Source: CAD feature listing. Evaluate the final solid. Frame: model axes, mm. Give positions to 0.01 mm unless a question says otherwise; leave off trailing zeros. Order: outer loops, then holes, each group sorted by start corner. A loop starts at its lowest first (then second) coordinate and runs counter-clockwise, first axis right, second up.
```python
from build123d import *

# Parameters (mm, degrees)
SKETCH1_W           = 100
SKETCH1_H           = 80
SKETCH1_R           = 2
BOSS_EXTRUDE1_DEPTH = 1


with BuildPart() as part:
    # Sketch1 → Boss-Extrude1 (new body)
    with BuildSketch(Plane.XY):
        Rectangle(SKETCH1_W, SKETCH1_H)
        with Locations((45, 36)):
            Circle(SKETCH1_R, mode=Mode.SUBTRACT)
        with Locations((-45, 36)):
            Circle(SKETCH1_R, mode=Mode.SUBTRACT)
        with Locations(Location((-45, -36, 0), (0, 0, 180))):
            Circle(SKETCH1_R, mode=Mode.SUBTRACT)
        with Locations(Location((45, -36, 0), (0, 0, 180))):
            Circle(SKETCH1_R, mode=Mode.SUBTRACT)
    extrude(amount=BOSS_EXTRUDE1_DEPTH)


solid = part.part
```
1) Draft query along Y for faces 1 (the flat face through (-1, 1, 1)), 2 (the cylindrical face through (-44.566, -34.048, 0.493)). Return one class per face: +Y half, -Y half, draft (parallel to the pull), parting line (faces both ways), or undercut.
Report:
face 1: draft
face 2: undercut
2) Material intervals for L1, parallel to X at y = -36, z = 0.65; L2, parallel to Y at x = 45, z = 0.7; L3, parallel to X at y = 37, z = 0.7, sorted ascending.
Report:
L1: x = -50 to -47, -43 to 43, 47 to 50
L2: y = -40 to -38, -34 to 34, 38 to 40
L3: x = -50 to -46.73, -43.27 to 43.27, 46.73 to 50
3) Pin query (flat end, axial travel): pin 1 (3 mm diameter, centred on x = -45, y = 36, fed in from +Z). Return the tip coordinate at first contact, or that it passes through.
Report:
pin 1: passes through
4) Section query B-B, the plane x = 45. Return the cut outline in (y, z).
Report:
outline: (-40, 0) - (-38, 0) - (-38, 1) - (-40, 1) - close; (-34, 0) - (34, 0) - (34, 1) - (-34, 1) - close; (38, 0) - (40, 0) - (40, 1) - (38, 1) - close
5) Section query A-A, the plane y = -36. Return the cut outline in (x, z).
Report:
outline: (-50, 0) - (-47, 0) - (-47, 1) - (-50, 1) - close; (-43, 0) - (43, 0) - (43, 1) - (-43, 1) - close; (47, 0) - (50, 0) - (50, 1) - (47, 1) - close
